CAD build for the part. Positions are in the model's coordinates, mm. Face numbers are marked on the shaded views. A direction names the side the tool comes from. Give positions to 0.01 mm unless a question says otherwise; leave off trailing zeros. Write each loop counter-clockwise with the first axis right and the second up, starting at its lowest first coordinate (ties: lowest second). Pieces come first, ordered by that corner, then holes. Notation, with made-up numbers: (-4.75, -30) - (22.25, -30) arc R19 cw to (22.25, -5) - close; hole circle Ø11 at (39.25, 71.25). An arc over 180 degrees is marked (long way). Put each result on its own line as item: value. Start each with the question number.
1. Cut at D-D on x = 24. List the corners of the cut face in (y, z).
2. Wall check: line 1 (X direction, y = -8.35, z = -45); line 2 (Z direction, x = 27, y = -9); line 3 (Y direction, x = 27, z = -16.5). Give the ranges that are in metal, low to high.
3. Cut at C-C on x = 8. List the corners of the cut face in (y, z), and give its area (3 significant figures).
4. Cut at A-A on y = -32.5. List the corners of the cut face in (x, z), and give its area (3 significant figures).
5. Drop flat-ended pins along their axis: pin 1 (1.5 mm diameter, centred on x = 0.5, z = -28, fed in from -Y); pin 2 (1 mm diameter, centred on x = 0.5, z = -11, fed in from +Y); pin 3 (8 mm diameter, centred on x = 16, y = -23, fed in from -Z); pin 4 (8 mm diameter, centred on y = -12, z = -27, fed in from +X). Give the stop position or say it passes through.
6. Cut at B-B on z = -32.3. List the corners of the cut face in (x, y).
7. Tool access for the marked faces 1 and 2: list every direction of +Z, -Z, +X, -X, +Y, -Y with a clear straight run to the whole face (end or side of a thin tool).
from build123d import *

# Parameters (mm, degrees)
SKETCH_1_W              = 32
SKETCH_1_H              = 40
EXTRUDE_1_DEPTH         = 32
SKETCH_2_W              = 45.589932218
SKETCH_2_H              = 35.821991612
CUT_EXTRUDE_1_DEPTH     = 72.582120673
HOLE_WIZARD_3_5_3_5_1_D = 3.5
FILLET_1_R              = 0.5
FILLET_3_R              = 2.5
CUT_EXTRUDE_3_REACH     = 69.439
SKETCH_9_W              = 2
SKETCH_9_H              = 15
EXTRUDE_2_DEPTH         = 20
CUT_EXTRUDE_4_DEPTH     = 64.780874876
CHAMFER_1_SIZE          = 15
FILLET_4_R              = 5


with BuildPart() as part:
    # 草图1 → 凸台-拉伸1 (new body)
    with BuildSketch(Plane(origin=(0, 0, 0), x_dir=(0, -1, 0), z_dir=(-1, 0, 0))):
        with Locations((24, -30)):
            Rectangle(SKETCH_1_W, SKETCH_1_H)
    extrude(amount=-EXTRUDE_1_DEPTH)

    # 草图2 → 切除-拉伸1 (cut, through all)
    with BuildSketch(Plane(origin=(32, 0, 0), x_dir=(0, 0, -1), z_dir=(1, 0, 0))):
        with Locations((34.794966109, -27.910995806)):
            Rectangle(SKETCH_2_W, SKETCH_2_H)
    extrude(amount=-CUT_EXTRUDE_1_DEPTH, mode=Mode.SUBTRACT)

    # Ø3.5 (3.5) 直径孔1 (through all)
    with Locations(Plane(origin=(0, -10, 0), x_dir=(-1, 0, 0), z_dir=(0, -1, 0))):
        with Locations((-5.002954744, 32.3), (-27, 45)):
            Hole(HOLE_WIZARD_3_5_3_5_1_D / 2)

    # 圆角1
    fillet_1_edges = [part.edges().sort_by_distance(p)[0] for p in [
        (16, -10, -12),
    ]]
    fillet(fillet_1_edges, radius=FILLET_1_R)

    # 圆角3
    fillet_3_edges = [part.edges().sort_by_distance(p)[0] for p in [
        (16, -8, -10),
    ]]
    fillet(fillet_3_edges, radius=FILLET_3_R)

    # 草图8 → 切除-拉伸3 (cut, up to next)
    with BuildSketch(Plane(origin=(0, -8, 0), x_dir=(1, 0, 0), z_dir=(0, 1, 0)), mode=Mode.PRIVATE) as cut_extrude_3_sk1:
        with BuildLine():
            ThreePointArc((3.487410287, 31.425), (10.472127202, 23.460456811), (19.973062925, 18.775113816))
            ThreePointArc((19.973062925, 18.775113816), (22.11636645, 20.012550683), (20.878929583, 22.155854208))
            ThreePointArc((20.878929583, 22.155854208), (12.602792204, 26.237193502), (6.5184992, 33.175))
            ThreePointArc((6.5184992, 33.175), (4.127954744, 33.815544457), (3.487410287, 31.425))
        make_face()
    cut_extrude_3_tool1 = extrude(cut_extrude_3_sk1.sketch, amount=-CUT_EXTRUDE_3_REACH, mode=Mode.PRIVATE) & part.part
    add(cut_extrude_3_tool1.solids().sort_by_distance((12.026611, -8, -25.486299))[0], mode=Mode.SUBTRACT)

    # 草图9 → 凸台-拉伸2 (add)
    with BuildSketch(Plane.ZY):
        with Locations((-11, -32.5)):
            Rectangle(SKETCH_9_W, SKETCH_9_H)
    extrude(amount=EXTRUDE_2_DEPTH)

    # 草图10 → 切除-拉伸4 (cut, through all)
    with BuildSketch(Plane(origin=(0, 0, -12), x_dir=(-1, 0, 0), z_dir=(0, 0, -1))):
        with BuildLine():
            Line((-15, -30.75), (15, -30.75))
            ThreePointArc((15, -30.75), (16.75, -32.5), (15, -34.25))
            Line((15, -34.25), (-15, -34.25))
            ThreePointArc((-15, -34.25), (-16.75, -32.5), (-15, -30.75))
        make_face()
    extrude(amount=-CUT_EXTRUDE_4_DEPTH, mode=Mode.SUBTRACT)

    # 倒角1
    chamfer_1_edges = [part.edges().sort_by_distance(p)[0] for p in [
        (32, -40, -11),
    ]]
    chamfer(chamfer_1_edges, length=CHAMFER_1_SIZE)

    # 圆角4
    fillet_4_edges = [part.edges().sort_by_distance(p)[0] for p in [
        (-20, -40, -11),
        (0, -25, -11),
        (-20, -25, -11),
        (0, -9, -50),
        (32, -9, -50),
    ]]
    fillet(fillet_4_edges, radius=FILLET_4_R)


solid = part.part
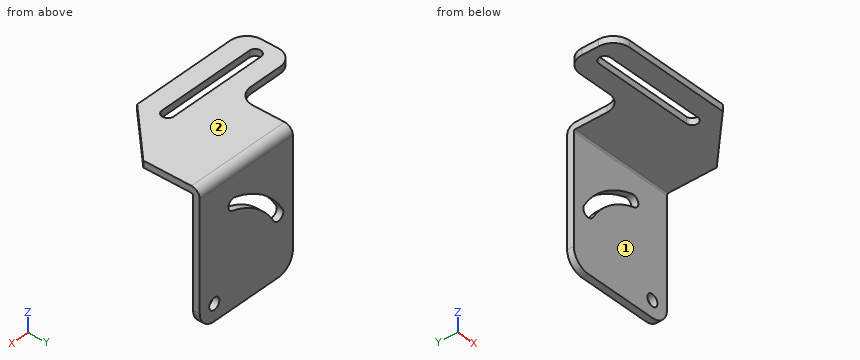
Report:
1. outline: (-33, -12) - (-10.5, -12) arc R0.5 cw to (-10, -12.5) - (-10, -50) - (-8, -50) - (-8, -12.5) arc R2.5 ccw to (-10.5, -10) - (-33, -10) - close
2. line 1: x = 0 to 25.25, 28.75 to 32
2. line 2: z = -50 to -46.75, -43.25 to -10.5
2. line 3: y = -10 to -8
3. outline: (-40, -12) - (-34.25, -12) - (-34.25, -10) - (-40, -10) - close; (-30.75, -12) - (-10.5, -12) arc R0.5 cw to (-10, -12.5) - (-10, -25.61) - (-8, -25.61) - (-8, -12.5) arc R2.5 ccw to (-10.5, -10) - (-30.75, -10) - close; (-10, -50) - (-8, -50) - (-8, -30.92) - (-10, -30.92) - close
3. area: 121 mm²
4. outline: (-20, -12) - (-16.75, -12) - (-16.75, -10) - (-20, -10) - close; (16.75, -12) - (24.5, -12) - (24.5, -10) - (16.75, -10) - close
4. area: 22.0 mm²
5. pin 1: stops at y = -10
5. pin 2: stops at y = -8.21
5. pin 3: stops at z = -12
5. pin 4: stops at x = 32
6. outline: (0, -10) - (3.25, -10) - (3.25, -8) - (0, -8) - close; (7.05, -10) - (32, -10) - (32, -8) - (7.05, -8) - close
7. face 1: -Z, +X, -X, -Y
7. face 2: +Z, +X, -X, +Y, -Y
